Source: three-view drawing plus pictorial views. Frame: mm from the lowest corner of the part. Give positions to 0.01 mm unless a question says otherwise; leave off trailing zeros. Loops run counter-clockwise (first coordinate to the right, second up) from the corner with the lowest first, then second, coordinate; pieces in that order, holes last. Notation, with made-up numbers: (56, 11) -> (78, 11) arc R22 ccw to (78, 43) -> close; hole circle Ø4 at (55.5, 13.5). An arc over 180 degrees is marked (long way). Answer in a Markdown table with one row per item. Add a question column.
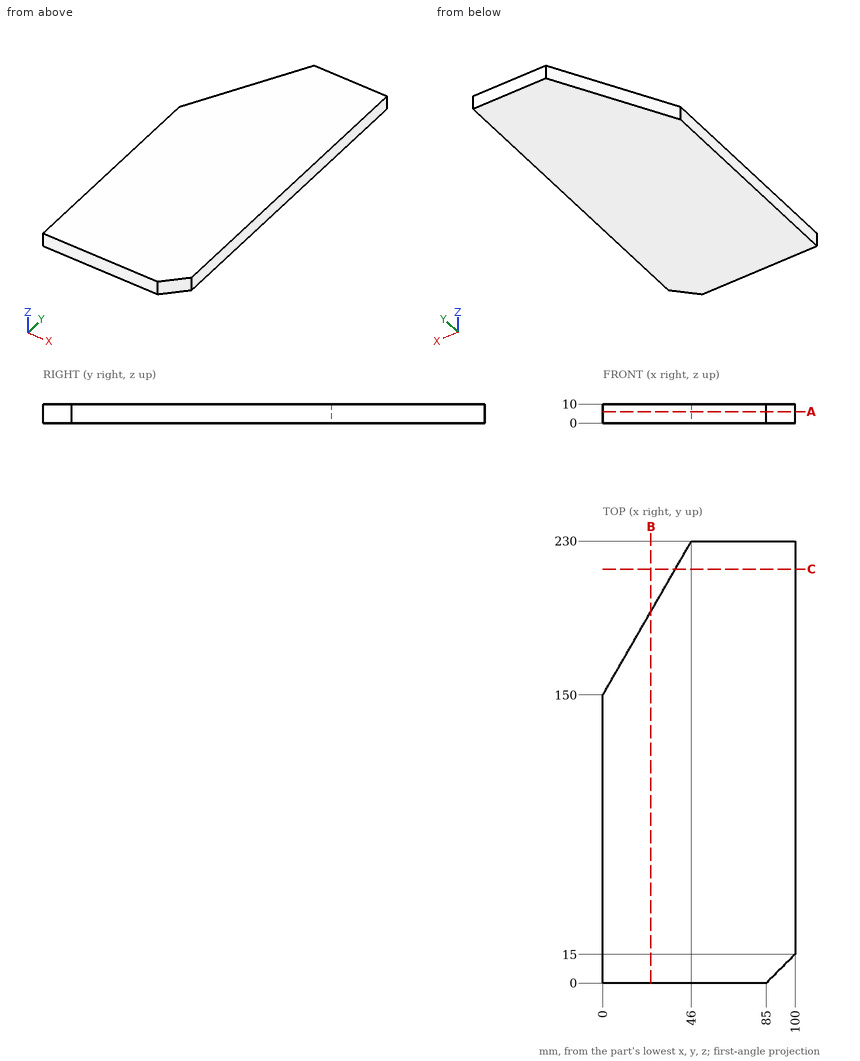
(1) Cut plane B-B on x = 25. Return the cut outline in (y, z).
(2) Cut plane C-C on y = 215.5. Return the cut outline in (x, z).
(3) Material intervals for line 1 along Y through (x, z) = (24, 3); line 2 along X through (y, z) = (186, 1.75); line 3 along Y through (x, z) = (14, 3.25), sorted ascending. Write a range as from..to.
(4) Cut plane A-A on z = 6. Return the cut outline in (x, y), then the cut area to 3 significant figures.
Answer list:
| question | item | result |
|---|---|---|
| 1 | outline | (0, 0) -> (193.48, 0) -> (193.48, 10) -> (0, 10) -> close |
| 2 | outline | (37.66, 0) -> (100, 0) -> (100, 10) -> (37.66, 10) -> close |
| 3 | line 1 | y = 0..191.74 |
| 3 | line 2 | x = 20.7..100 |
| 3 | line 3 | y = 0..174.35 |
| 4 | outline | (0, 0) -> (85, 0) -> (100, 15) -> (100, 230) -> (46, 230) -> (0, 150) -> close |
| 4 | area | 21,000 mm² |
